The model under review builds one solid part; all positions refer to its coordinate system, in mm. Face numbers are marked on the shaded views. A direction names the side the tool comes from. Coordinates: 2 decimals unless noted, no trailing zeros. Loops run counter-clockwise (first coordinate to the right, second up) from the corner with the lowest first, then second, coordinate; pieces in that order, holes last. Notation, with made-up numbers: M 10,68.5 L 58,68.5 A30 ccw 58,97.5 Z; hole C 19.25,-36.75 d3. An arc over 180 degrees is marked long. Return JSON: item names as keys, results as strings.
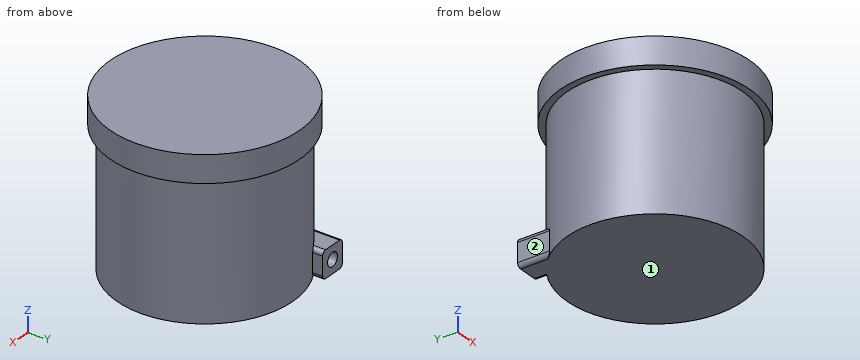
```python
from build123d import *

# Parameters (mm, degrees)
SKETCH1_R           = 65
BOSS_EXTRUDE1_DEPTH = 100
SKETCH2_R           = 70
BOSS_EXTRUDE2_DEPTH = 20
SKETCH4_W           = 20
SKETCH4_H           = 24.089012679
BOSS_EXTRUDE4_DEPTH = 20
SKETCH5_R           = 5
CUT_EXTRUDE1_DEPTH  = 15
FILLET1_R           = 3


with BuildPart() as part:
    # Sketch1 → Boss-Extrude1 (new body)
    with BuildSketch(Plane.XY):
        Circle(SKETCH1_R)
    extrude(amount=BOSS_EXTRUDE1_DEPTH)

    # Sketch2 → Boss-Extrude2 (add)
    with BuildSketch(Plane.XY.offset(100)):
        Circle(SKETCH2_R)
    extrude(amount=BOSS_EXTRUDE2_DEPTH)

    # Sketch4 → Boss-Extrude4 (add)
    with BuildSketch(Plane(origin=(0, 0, 0), x_dir=(-1, 0, 0), z_dir=(0, 0, -1))):
        with Locations((40, 52.95549366)):
            Rectangle(SKETCH4_W, SKETCH4_H)
    extrude(amount=-BOSS_EXTRUDE4_DEPTH)

    # Sketch5 → Cut-Extrude1 (cut)
    with BuildSketch(Plane(origin=(0, 65, 0), x_dir=(1, 0, 0), z_dir=(0, 1, 0))):
        with Locations(Location((-40, -10, 0), (0, 0, 270))):
            Circle(SKETCH5_R)
    extrude(amount=-CUT_EXTRUDE1_DEPTH, mode=Mode.SUBTRACT)

    # Fillet1
    fillet1_edges = [part.edges().sort_by_distance(p)[0] for p in [
        (-30, 61.331406487, 20),
        (-50, 53.266559657, 20),
        (-30, 61.331406487, 0),
        (-50, 53.266559657, 0),
    ]]
    fillet(fillet1_edges, radius=FILLET1_R)


solid = part.part
```
1. Machinability: for the marked faces 1 and 2, which of the approach directions +Z, -Z, +X, -X, +Y, -Y give a long, thin tool a straight path to every point of the face, cutting with its end or side? Answer none if there is none.
Check values:
{"face 1": "-Z, +X, -X, +Y, -Y", "face 2": "-Z, -X, +Y"}
2. Add section B-B on x = 0. Give the boundary of the cut face in (y, z).
Check values:
{"outline": "M -70,100 L -65,100 L -65,0 L 65,0 L 65,100 L 70,100 L 70,120 L -70,120 Z"}
3. To check wall thickness, follow line 1 (X direction, y = 59.5, z = 10); line 2 (Y direction, x = 46.5, z = 110); line 3 (X direction, y = -19, z = 115). State the ranges of each line that lie inside material, in increasing order.
Check values:
{"line 1": "-50 to -45, -35 to -30, -26.17 to 26.17", "line 2": "-52.32 to 52.32", "line 3": "-67.37 to 67.37"}
4. Add section D-D on z = 65.5. Give the boundary of the cut face in (x, y), plus the area to 3 significant figures.
Check values:
{"outline": "C 0,0 d130", "area": "13,300 mm²"}
5. Add section A-A on z = 10. Give the boundary of the cut face in (x, y), plus the area to 3 significant figures.
Check values:
{"outline": "M -50,41.53 A65 ccw long -30,57.66 L -30,65 L -35,65 L -35,50 L -45,50 L -45,65 L -50,65 Z", "area": "13,400 mm²"}
6. Add section C-C on x = -40. Give the boundary of the cut face in (y, z), plus the area to 3 significant figures.
Check values:
{"outline": "M -57.45,100 L -51.23,100 L -51.23,0 L 65,0 L 65,5 L 50,5 L 50,15 L 65,15 L 65,20 L 51.23,20 L 51.23,100 L 57.45,100 L 57.45,120 L -57.45,120 Z", "area": "12,700 mm²"}
7. Insertion check: pin 1 Ø4 at (x, y) = (-43.5, 58) entering from +Z; pin 2 Ø11 at (x, z) = (-42.5, 9.5) entering from +Y; pin 3 Ø15.5 at (y, z) = (59, 7.5) entering from -X. Each pin has a flat end and moves straight along its axis. Give the tip position at first contact, or say it passes through.
Check values:
{"pin 1": "z = 20", "pin 2": "y = 65", "pin 3": "x = -50"}
